Geometry check sheet. Reference: drawing and pictorial views, mm from the part's lowest x, y, z. A direction names the side the tool comes from. Round coordinates to 2 decimals unless told otherwise and drop trailing zeros. Write each loop counter-clockwise with the first axis right and the second up, starting at its lowest first coordinate (ties: lowest second). Pieces come first, ordered by that corner, then holes. Notation, with made-up numbers: (-40, 35) - (2, 35) arc R30 ccw to (2, 70) - close; hole circle Ø3 at (58.25, -23). An arc over 180 degrees is marked (long way). Use one line per item in the form item = value. Start each with the question number.
1) Gauge pin test, flat ends, axial feed: P1, Ø11, axis at y = 33.5, z = 4.5, coming from the +X side; P2, Ø3, axis at y = 65, z = 43.5, coming from the +X side; P3, Ø25, axis at x = 306, z = 34, coming from the -Y side. Record the tip position at first contact, or that the pin passes through.
2) Section check B-B (y = 184). Record the boundary of the cut face in (x, z), then the cut area to 3 significant figures.
3) Section check A-A (z = 19). Record the boundary of the cut face in (x, y).
4) Set-up check for the marked faces 4 and 5: record each of +Z, -Z, +X, -X, +Y, -Y from which the full face is reachable in a straight line by a thin tool's end or side.
5) Draft check along Y on the marked faces 1, 2 and 3. Enter one of: +Y half, -Y half, draft (parallel to the pull), parting line (faces both ways), or undercut.
6) Scan lines: probe 1 along Y at (x, z) = (565, 5); probe 2 along Y at (x, z) = (152.5, 22); probe 3 along Y at (x, z) = (80, 42). Record each from-to range of solid material in increasing order.
7) Section check C-C (x = 537.5). Record the boundary of the cut face in (y, z), then the cut area to 3 significant figures.
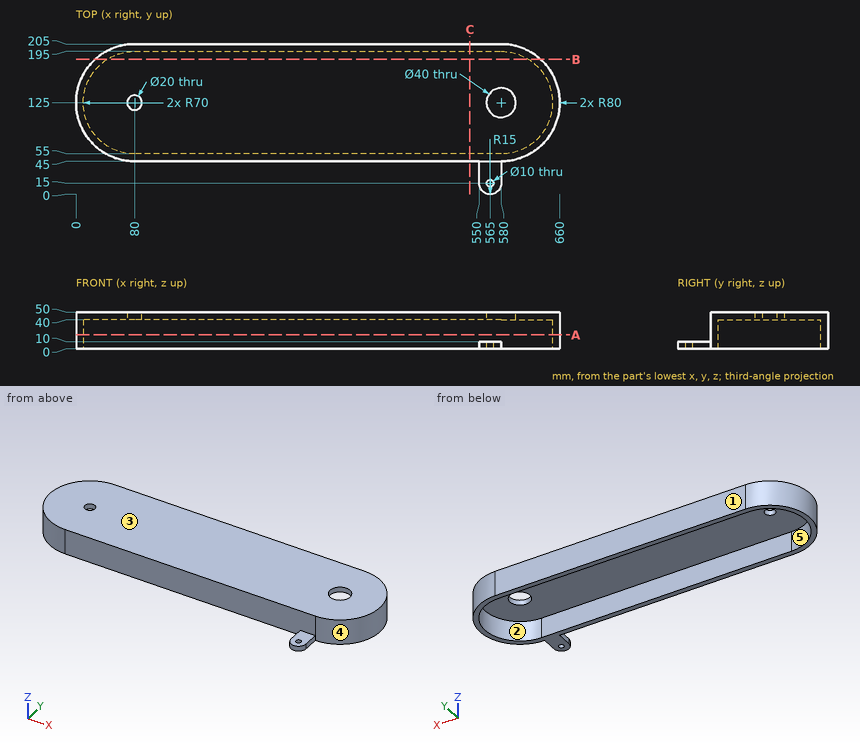
Results are:
q1.P1 = 580
q1.P2 = 634.57
q1.P3 = 45
q2.outline = (25.97, 0) - (42.33, 0) - (42.33, 40) - (617.67, 40) - (617.67, 0) - (634.03, 0) - (634.03, 50) - (25.97, 50) - close
q2.area = 7,390 mm²
q3.outline = (80, 45) - (580, 45) arc R80 ccw to (580, 205) - (80, 205) arc R80 ccw to start; hole (80, 55) - (580, 55) arc R70 ccw to (580, 195) - (80, 195) arc R70 ccw to start
q4.face_4 = +Z, -Z, +X
q4.face_5 = -Z
q5.face_1 = +Y half
q5.face_2 = undercut
q5.face_3 = draft
q6.probe_1 = 0 to 10, 20 to 55, 195 to 205
q6.probe_2 = 45 to 55, 195 to 205
q6.probe_3 = 45 to 115, 135 to 205
q7.outline = (45, 0) - (55, 0) - (55, 40) - (195, 40) - (195, 0) - (205, 0) - (205, 50) - (45, 50) - close
q7.area = 2,400 mm²
